Build history of the part. All positions in model axes, mm. A direction names the side the tool comes from. Coordinates: 2 decimals unless noted, no trailing zeros. Write each loop counter-clockwise with the first axis right and the second up, starting at its lowest first coordinate (ties: lowest second). Pieces come first, ordered by that corner, then holes. Notation, with made-up numbers: (81, -18.75) -> (137, -18.75) arc R31 ccw to (137, 8.25) -> close; hole circle Ø1 at (-32.5, 77). An arc over 180 degrees is marked (long way). Write each question's results on one line, items separated by ' | '. Start each with the question number.
Q1. Drill centre lines: line 1 (Y direction, x = 27, z = -2.5); line 2 (Z direction, x = -20, y = 102); line 3 (Y direction, x = 31.5, z = -0.5). Where is each one in solid material? Low to high.
Q2. Two-plate mould, pull along X, no slides. Class faces 1 (the face through (4, 178, 26)), 2 (the face through (0, 151, 27)), 3 (the face through (39.996, 5.07, -0.531)), 4 (the face through (0, 200, -1)): released by +X, released by -X, zero draft, split by the parting line, or undercut.
Q3. Saw through at A-A on z = 0. Give the cut face in (x, y), and give its area (3 significant figures).
Q4. Drop flat-ended pins along their axis: pin 1 Ø3 at (y, z) = (175, -3) entering from -X; pin 2 Ø1.9 at (y, z) = (178.5, 25.5) entering from -X; pin 3 Ø4 at (x, y) = (28, 123.5) entering from +Z. Give the stop position or say it passes through.
Q5. Tool access for faces 5 (the face through (-4, 177, 26)), 6 (the face through (-18, 10, -27)), 7 (the face through (-1, 0, 0)): list every direction of +Z, -Z, +X, -X, +Y, -Y with a clear straight run to the whole face (end or side of a thin tool).
Q6. Saw through at C-C on y = 61.5. Give the cut face in (x, z), and give its area (3 significant figures).
Q7. Saw through at B-B on y = 187.5. Give the cut face in (x, z).
from build123d import *

# Parameters (mm, degrees)
SKETCH2_OUTSIDE_W   = 127.956
SKETCH2_OUTSIDE_H   = 127.956
SKETCH2_OUTSIDE_W_2 = 130
SKETCH2_OUTSIDE_H_2 = 65
CUT_EXTRUDE1_DEPTH  = 10
CUT_EXTRUDE2_REACH  = 213.642
CHAMFER1_SIZE       = 1
FILLET2_R           = 2


with BuildPart() as part:
    # Sketch1 → Revolve1 (revolve)
    with BuildSketch(Plane.XY, mode=Mode.PRIVATE) as revolve1_sk:
        Polygon((0, 0), (40, 0), (40, 10), (30, 10), (30, 155), (28, 155), (28, 200), (0, 200), align=None)
    revolve(revolve1_sk.sketch.rotate(Axis((0, 0, 0), (0, -1, 0)), 90), axis=Axis((0, 0, 0), (0, -1, 0)))

    # Sketch2 outside → Cut-Extrude1 (cut)
    with BuildSketch(Plane(origin=(0, 0, 0), x_dir=(1, 0, 0), z_dir=(0, 1, 0))):
        Rectangle(SKETCH2_OUTSIDE_W, SKETCH2_OUTSIDE_H)
        Rectangle(SKETCH2_OUTSIDE_W_2, SKETCH2_OUTSIDE_H_2, mode=Mode.SUBTRACT)
    extrude(amount=CUT_EXTRUDE1_DEPTH, mode=Mode.SUBTRACT)

    # Sketch3 → Cut-Extrude2 (cut, up to next)
    with BuildSketch(Plane.XY.offset(24), mode=Mode.PRIVATE) as cut_extrude2_sk1:
        with BuildLine():
            Line((4, 200), (4, 155))
            ThreePointArc((4, 155), (0, 151), (-4, 155))
            Line((-4, 155), (-4, 200))
            ThreePointArc((-4, 200), (0, 204), (4, 200))
        make_face()
    cut_extrude2_tool1 = extrude(cut_extrude2_sk1.sketch, amount=CUT_EXTRUDE2_REACH, mode=Mode.PRIVATE) & part.part
    add(cut_extrude2_tool1.solids().sort_by_distance((0, 177.5, 24))[0], mode=Mode.SUBTRACT)

    # Chamfer1
    chamfer1_edges = [part.edges().sort_by_distance(p)[0] for p in [
        (0, 200, -28),
    ]]
    chamfer(chamfer1_edges, length=CHAMFER1_SIZE)

    # Fillet2
    fillet2_edges = [part.edges().sort_by_distance(p)[0] for p in [
        (0, 10, -30),
    ]]
    fillet(fillet2_edges, radius=FILLET2_R)


solid = part.part
Returned:
1) line 1: y = 0 to 199.88 | line 2: z = -22.36 to 22.36 | line 3: y = 0 to 10.06
2) face 1: undercut | face 2: undercut | face 3: released by +X | face 4: zero draft
3) outline: (-40, 0) -> (40, 0) -> (40, 10) -> (32, 10) arc R2 cw to (30, 12) -> (30, 155) -> (28, 155) -> (28, 199) -> (27, 200) -> (-27, 200) -> (-28, 199) -> (-28, 155) -> (-30, 155) -> (-30, 12) arc R2 cw to (-32, 10) -> (-40, 10) -> close | area: 12,000 mm2
4) pin 1: stops at x = -27.96 | pin 2: stops at x = -13.46 | pin 3: stops at z = 14.97
5) face 5: +Z, +Y | face 6: +Y | face 7: +Z, -Z, +X, -X, -Y
6) outline: circle Ø60 at (0, 0) | area: 2,830 mm2
7) outline: (-4, 24) -> (-4, 27.71) arc R28 ccw (long way) to (4, 27.71) -> (4, 24) -> close
